```python
from build123d import *

# Parameters (mm, degrees)
SKETCH_3_W          = 2.4
SKETCH_3_H          = 3.7
EXTRUDE_1_DEPTH     = 5
CUT_EXTRUDE_START   = -10
SKETCH_5_R          = 16
CUT_EXTRUDE_1_DEPTH = 10
SKETCH_6_R          = 17.5
SKETCH_6_R_2        = 13.5
EXTRUDE_2_DEPTH     = 7.5


with BuildPart() as part:
    # 草图2 → Revolve 1 (revolve)
    with BuildSketch(Plane.XY, mode=Mode.PRIVATE) as revolve_1_sk:
        Polygon((-16, 26.2), (-16, -26.35), (-20.8, -26.35), (-20.8, 26.35), (-16.15, 26.35), align=None)
    revolve(revolve_1_sk.sketch.rotate(Axis((0, -26.35, 0), (0, 1, 0)), 270), axis=Axis((0, -26.35, 0), (0, 1, 0)))

    # 草图3 → Revolve 1 2 (revolve)
    with BuildSketch(Plane.XY, mode=Mode.PRIVATE) as revolve_1_2_sk:
        with Locations((-14.8, 1.85)):
            Rectangle(SKETCH_3_W, SKETCH_3_H)
    revolve(revolve_1_2_sk.sketch.rotate(Axis((0, -26.35, 0), (0, 1, 0)), 270), axis=Axis((0, -26.35, 0), (0, 1, 0)))

    # 草图4 → 凸台-拉伸1 (add, symmetric)
    with BuildSketch(Plane(origin=(0, 0, 0), x_dir=(1, 0, 0), z_dir=(0, 1, 0))):
        Polygon((23.124383018, 6.489702871), (5.94194396, 23.271154576), (-17.182439058, 16.781451705), (-23.124383018, -6.489702871), (-5.94194396, -23.271154576), (17.182439058, -16.781451705), align=None)
    extrude(amount=EXTRUDE_1_DEPTH, both=True)

    # 草图5 → 切除-拉伸1 (cut)
    with BuildSketch(Plane(origin=(0, 5, 0), x_dir=(1, 0, 0), z_dir=(0, 1, 0)).offset(CUT_EXTRUDE_START)):
        with Locations(Location((0, 0, 0), (0, 0, 90))):
            Circle(SKETCH_5_R)
    extrude(amount=CUT_EXTRUDE_1_DEPTH, mode=Mode.SUBTRACT)

    # 草图6 → 凸台-拉伸2 (add, symmetric)
    with BuildSketch(Plane(origin=(0, 0, 0), x_dir=(1, 0, 0), z_dir=(0, 1, 0))):
        Circle(SKETCH_6_R)
        with Locations(Location((0, 0, 0), (0, 0, 270))):
            Circle(SKETCH_6_R_2, mode=Mode.SUBTRACT)
    extrude(amount=EXTRUDE_2_DEPTH, both=True)


solid = part.part
```
The listing builds one solid part. Answer for the finished solid, in the listing's coordinates (mm). A direction names the side the tool comes from. Round coordinates to 2 decimals unless told otherwise and drop trailing zeros. Loops run counter-clockwise (first coordinate to the right, second up) from the corner with the lowest first, then second, coordinate; pieces in that order, holes last.
Q1. Section D-D, the plane x = 19 is taken. Determine the outline of the cut face in (y, z), then the cut area to 3 significant figures.
Q2. Given pin 1 Ø6 at (x, y) = (-13, -11) entering from -Z; pin 2 Ø1.5 at (x, y) = (11, -20) entering from -Z; pin 3 Ø3 at (y, z) = (17.5, -13) entering from -X; pin 4 Ø19 at (x, z) = (0, 0) entering from -Y, each flat-ended and moving along its own axis, determine where each tip first touches the part or whether it passes through.
Q3. Section A-A, the plane y = 4 is taken. Determine the outline of the cut face in (x, z), then the cut area to 3 significant figures.
Q4. Section B-B, the plane x = 0 is taken. Determine the outline of the cut face in (y, z).
Q5. Which of the six approach directions +Z, -Z, +X, -X, +Y, -Y give full straight-line access (tool end or side, diameter ignored) to faces 4 (the face through (15.62, -17.06, 3.47)), 5 (the face through (16, 5, 15)), 6 (the face through (-6.25, 15.82, -19.84))?
Q6. Find the intervals of material crossed by line 1 (X direction, y = -22, z = 0); line 2 (Y direction, x = 15, z = 2); line 3 (Z direction, x = 1.5, y = -12.5), in increasing order.
Q7. For a pull along Z with two mould halves and no side action, classify faces 1 (the face through (20.11, 0.07, 5.31)), 2 (the face through (-7, 7.5, 12)), 3 (the face through (21, -5, -6)) as released by +Z, released by -Z, zero draft, split by the parting line, or undercut.
Q8. Section C-C, the plane z = 0 is taken. Determine the outline of the cut face in (x, y).
Completed:
1. outline: (-26.35, -8.46) - (-5, -8.46) - (-5, -10.52) - (5, -10.52) - (5, -8.46) - (26.35, -8.46) - (26.35, 8.46) - (5, 8.46) - (5, 9.66) - (-5, 9.66) - (-5, 8.46) - (-26.35, 8.46) - close
1. area: 925 mm2
2. pin 1: stops at z = -18.24
2. pin 2: stops at z = -18.1
2. pin 3: stops at x = -17.33
2. pin 4: passes through
3. outline: (-23.12, 6.49) - (-17.18, -16.78) - (5.94, -23.27) - (23.12, -6.49) - (17.18, 16.78) - (-5.94, 23.27) - close; hole circle Ø27 at (0, 0)
3. area: 926 mm2
4. outline: (-26.35, -20.8) - (-5, -20.8) - (-5, -21.6) - (5, -21.6) - (5, -20.8) - (26.35, -20.8) - (26.35, -16.15) - (26.2, -16) - (7.5, -16) - (7.5, -13.5) - (-7.5, -13.5) - (-7.5, -16) - (-26.35, -16) - close; (-26.35, 16) - (-7.5, 16) - (-7.5, 13.5) - (7.5, 13.5) - (7.5, 16) - (26.2, 16) - (26.35, 16.15) - (26.35, 20.8) - (5, 20.8) - (5, 21.6) - (-5, 21.6) - (-5, 20.8) - (-26.35, 20.8) - close
5. face 4: -Y
5. face 5: +Z, +X, +Y
5. face 6: +Y
6. line 1: x = -20.8 to -16, 16 to 20.8
6. line 2: y = -7.5 to 7.5
6. line 3: z = -20.75 to -15.93, 15.93 to 20.75
7. face 1: released by +Z
7. face 2: undercut
7. face 3: zero draft
8. outline: (-21.47, -5) - (-20.8, -5) - (-20.8, -26.35) - (-16, -26.35) - (-16, -7.5) - (-13.5, -7.5) - (-13.5, 7.5) - (-16, 7.5) - (-16, 26.2) - (-16.15, 26.35) - (-20.8, 26.35) - (-20.8, 5) - (-21.47, 5) - close; (13.5, -7.5) - (16, -7.5) - (16, -26.35) - (20.8, -26.35) - (20.8, -5) - (21.47, -5) - (21.47, 5) - (20.8, 5) - (20.8, 26.35) - (16.15, 26.35) - (16, 26.2) - (16, 7.5) - (13.5, 7.5) - close
